Read the model definition and answer for the solid it produces. Units are mm, in the model's axes. A direction names the side the tool comes from. Give positions to 0.01 mm unless a question says otherwise; leave off trailing zeros. Loops run counter-clockwise (first coordinate to the right, second up) from the corner with the lowest first, then second, coordinate; pieces in that order, holes last.
(1) Find section B-B, the plane y = -102.5. Write down the section's boundary in (x, z), then the cut area to 3 significant figures.
(2) Which of the six approach directions +Z, -Z, +X, -X, +Y, -Y give full straight-line access (tool end or side, diameter ignored) to faces 4 (the face through (6, -14, 32)), 5 (the face through (3, -46, 33)), 6 (the face through (6, -81, 32))?
(3) Find section D-D, the plane y = -78.5. Write down the section's boundary in (x, z), then the cut area to 3 significant figures.
(4) Straight lines are drawn through the part: probe 1 along Y at (x, z) = (28, 3.9); probe 2 along Y at (x, z) = (-14.5, 38); probe 3 along Z at (x, y) = (13.5, -8). For each, find the intervals that lie inside material, in ascending order.
(5) Each of these flat-tipped pins is pushed along its axis until it touches: P1, Ø1.8, axis at x = 4, z = 30, coming from the -Y side; P2, Ø2, axis at y = -97.5, z = 33.5, coming from the -X side; P3, Ø4, axis at y = -72, z = 17.5, coming from the +X side; P4, Ø8, axis at x = -5, y = -64, coming from the -Z side. Where does it stop, or does it pass through?
(6) Find section A-A, the plane z = 27.5. Write down the section's boundary in (x, y), then the cut area to 3 significant figures.
(7) Determine the mould class of faces 1 (the face through (12, -49, 0)), 2 (the face through (22, -18, 3)), 3 (the face through (3, -33, 19)) for opening direction Z: pulls with the +Z half, pulls with the -Z half, needs draft (parallel to the pull), parting line crosses it, or undercut.
(8) Find section C-C, the plane z = 14. Write down the section's boundary in (x, y), then the cut area to 3 significant figures.
```python
from build123d import *

# Parameters (mm, degrees)
BACK_PLATE_PROFILE_R   = 6
BACK_PLATE_6MM_DEPTH   = 6
SIDE_FLANGE_PROFILE_R  = 10
SIDE_FLANGE_6MM_DEPTH  = 6
GUSSET_RIB_10MM_REACH  = 93.258
GUSSET_RIB_PATH_WALL_W = 238.92163478
GUSSET_RIB_PATH_WALL_H = 10
CRADLE_SADDLE_REACH    = 132.629


with BuildPart() as part:
    # Back Plate Profile → Back Plate 6mm (new body)
    with BuildSketch(Plane.XY):
        with BuildLine():
            Line((0, 0), (6, 0))
            Line((6, 0), (30.967735953, -6.372767169))
            ThreePointArc((30.967735953, -6.372767169), (39.129158997, -13.512036094), (38.203470161, -24.315789474))
            ThreePointArc((38.203470161, -24.315789474), (34.310988843, -38), (38.203470161, -51.684210526))
            ThreePointArc((38.203470161, -51.684210526), (39.723835971, -55.440376954), (39.907334521, -59.488416815))
            Line((39.907334521, -59.488416815), (34.907334521, -99.488416815))
            ThreePointArc((34.907334521, -99.488416815), (30.941630759, -106.99613811), (23, -110))
            Line((23, -110), (0, -110))
            Line((0, -110), (0, 0))
        make_face()
        with Locations((23, -98)):
            Circle(BACK_PLATE_PROFILE_R, mode=Mode.SUBTRACT)
        with Locations((28, -58)):
            Circle(BACK_PLATE_PROFILE_R, mode=Mode.SUBTRACT)
        with Locations((28, -18)):
            Circle(BACK_PLATE_PROFILE_R, mode=Mode.SUBTRACT)
    extrude(amount=BACK_PLATE_6MM_DEPTH)

    # Side Flange Profile → Side Flange 6mm (add)
    with BuildSketch(Plane(origin=(0, 0, 0), x_dir=(0, 0, -1), z_dir=(1, 0, 0))):
        with BuildLine():
            Line((0, 0), (-58, 0))
            Line((-58, 0), (-58, -68))
            Line((-58, -68), (-43.858565284, -98.428947708))
            ThreePointArc((-43.858565284, -98.428947708), (-36.478390759, -106.860886011), (-25.721508176, -110))
            Line((-25.721508176, -110), (-5.721508176, -110))
            Line((-5.721508176, -110), (0, -110))
            Line((0, -110), (0, 0))
        make_face()
        with Locations((-25.721508176, -90)):
            Circle(SIDE_FLANGE_PROFILE_R, mode=Mode.SUBTRACT)
        with BuildLine():
            Line((-40, -46), (-25, -46))
            ThreePointArc((-25, -46), (-20.757359313, -44.242640687), (-19, -40))
            Line((-19, -40), (-19, -26))
            ThreePointArc((-19, -26), (-20.757359313, -21.757359313), (-25, -20))
            Line((-25, -20), (-40, -20))
            ThreePointArc((-40, -20), (-44.242640687, -21.757359313), (-46, -26))
            Line((-46, -26), (-46, -40))
            ThreePointArc((-46, -40), (-44.242640687, -44.242640687), (-40, -46))
        make_face(mode=Mode.SUBTRACT)
    extrude(amount=SIDE_FLANGE_6MM_DEPTH)

    # Gusset Rib Path wall → Gusset Rib 10mm (add, up to next)
    with BuildSketch(Plane(origin=(14, -58, 32), x_dir=(0.294085848838, 0, -0.955779008722), z_dir=(-0.955779008722, 0, -0.294085848838)), mode=Mode.PRIVATE) as gusset_rib_10mm_sk1:
        Rectangle(GUSSET_RIB_PATH_WALL_W, GUSSET_RIB_PATH_WALL_H)
    gusset_rib_10mm_tool1 = extrude(gusset_rib_10mm_sk1.sketch, amount=GUSSET_RIB_10MM_REACH, mode=Mode.PRIVATE) - part.part
    add(gusset_rib_10mm_tool1.solids().sort_by_distance((14, -58, 32))[0])

    # Cradle Saddle: up to this face of the body (flat: up to its plane)
    cradle_saddle_end = Plane(part.part.faces().sort_by_distance((17.427592869, -55.606488982, 0))[0])
    # Cradle Saddle Profile → Cradle Saddle (add, up to the picked face)
    with BuildSketch(Plane.XY.offset(58), mode=Mode.PRIVATE) as cradle_saddle_sk1:
        with BuildLine():
            Line((-33, 0), (-33, 11))
            Line((-33, 11), (-28, 11))
            Line((-28, 11), (-28, 0))
            ThreePointArc((-28, 0), (-14, -14), (0, 0))
            Line((0, 0), (0, -33))
            ThreePointArc((0, -33), (-4.100505063, -23.100505063), (-14, -19))
            ThreePointArc((-14, -19), (-27.435028843, -13.435028843), (-33, 0))
        make_face()
    cradle_saddle_tool1 = split(extrude(cradle_saddle_sk1.sketch, amount=-CRADLE_SADDLE_REACH, mode=Mode.PRIVATE), bisect_by=cradle_saddle_end, keep=Keep.BOTH, mode=Mode.PRIVATE)
    add(cradle_saddle_tool1.solids().sort_by(Axis((-27.04612, -13.04612, 58), (0, 0, -1)))[0])


solid = part.part
```
Entries:
1. outline: (0, 0) - (19.03, 0) - (19.03, 6) - (6, 6) - (6, 41.33) - (0, 41.33) - close; (26.97, 0) - (34.12, 0) - (34.12, 6) - (26.97, 6) - close
1. area: 369 mm2
2. face 4: +Z, +X, +Y
2. face 5: +X, -X
2. face 6: +Z, +X, -Y
3. outline: (0, 0) - (37.53, 0) - (37.53, 6) - (6, 6) - (6, 53.12) - (0, 53.12) - close
3. area: 508 mm2
4. probe 1: y = -108.91 to -101.32, -94.68 to -64, -52 to -24, -12 to -5.62
4. probe 2: y = -18.99 to -13.99
4. probe 3: z = 0 to 6
5. P1: stops at y = -109.71
5. P2: stops at x = 0
5. P3: stops at x = 6
5. P4: passes through
6. outline: (-33, 0) arc R19 ccw to (-14, -19) arc R14 cw to (0, -33) - (0, -20) - (6, -20) - (6, 0) - (0, 0) arc R14 cw to (-28, 0) - (-28, 11) - (-33, 11) - close; (0, -109.92) - (6, -109.92) - (6, -99.84) - (0, -99.84) - close; (0, -80.16) - (6, -80.16) - (6, -63) - (15.38, -63) - (15.38, -53) - (6, -53) - (6, -46) - (0, -46) - close
6. area: 818 mm2
7. face 1: pulls with the -Z half
7. face 2: needs draft
7. face 3: undercut
8. outline: (-33, 0) arc R19 ccw to (-14, -19) arc R14 cw to (0, -33) - (0, -110) - (6, -110) - (6, -63) - (19.54, -63) - (19.54, -53) - (6, -53) - (6, 0) - (0, 0) arc R14 cw to (-28, 0) - (-28, 11) - (-33, 11) - close
8. area: 1,130 mm2
